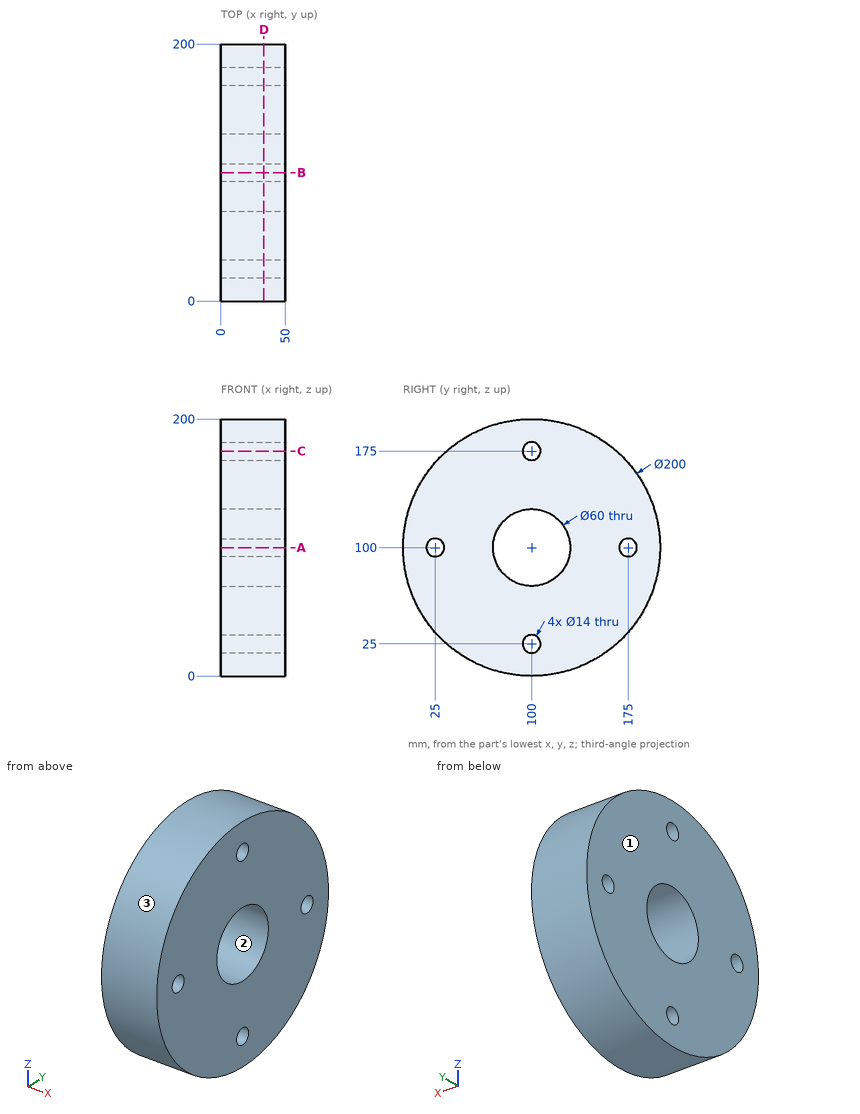
Study the drawing (mm; zero at the part's minimum x, y, z) and answer. Give positions to 0.01 mm unless a question says otherwise; leave off trailing zeros. Loops run counter-clockwise (first coordinate to the right, second up) from the corner with the lowest first, then second, coordinate; pieces in that order, holes last. Notation, with made-up numbers: M -22.5,54 L -18.5,54 A30 ccw -18.5,80 Z; hole C 81,70 d10. An arc over 180 degrees is marked long. Use CSV: the item, a comma, the result in double quotes.
1) Consider L1, parallel to Y at x = 10.5, z = 109; L2, parallel to Y at x = 42.5, z = 104.5; L3, parallel to Y at x = 3, z = 169. Determine where each line is inside the solid, lowest interval first.
Answer:
L1,"0.41 to 71.38, 128.62 to 199.59"
L2,"0.1 to 19.64, 30.36 to 70.34, 129.66 to 169.64, 180.36 to 199.9"
L3,"27.62 to 96.39, 103.61 to 172.38"
2) Find section C-C on z = 175. Write down the section's boundary in (x, y).
Answer:
outline,"M 0,33.86 L 50,33.86 L 50,93 L 0,93 Z; M 0,107 L 50,107 L 50,166.14 L 0,166.14 Z"
3) Given P1, Ø8, axis at x = 30, z = 178, coming from the +Y side; P2, Ø4, axis at x = 32.5, y = 106.5, coming from the -Z side; P3, Ø1.5, axis at x = 31, z = 118, coming from the +Y side, each flat-ended and moving along its own axis, determine where each tip first touches the part or whether it passes through.
Answer:
P1,"y = 167.26"
P2,"z = 0.1"
P3,"y = 198.5"
4) Find section D-D on x = 33.5. Write down the section's boundary in (y, z).
Answer:
outline,"C 100,100 d200; hole C 25,100 d14; hole C 100,100 d60; hole C 100,25 d14; hole C 100,175 d14; hole C 175,100 d14"
5) Find section A-A on z = 100. Write down the section's boundary in (x, y).
Answer:
outline,"M 0,0 L 50,0 L 50,18 L 0,18 Z; M 0,32 L 50,32 L 50,70 L 0,70 Z; M 0,130 L 50,130 L 50,168 L 0,168 Z; M 0,182 L 50,182 L 50,200 L 0,200 Z"
6) Determine the mould class of the marked faces 1, 2 and 3 for opening direction Z: released by +Z, released by -Z, zero draft, split by the parting line, or undercut.
Answer:
face 1,"zero draft"
face 2,"undercut"
face 3,"split by the parting line"
